```python
from build123d import *

# Parameters (mm, degrees)
BOSS_EXTRUDE1_DEPTH = 14
SKETCH3_W           = 2.1
SKETCH3_H           = 12.5


with BuildPart() as part:
    # Sketch1 → Boss-Extrude1 (new body)
    with BuildSketch(Plane.XY):
        with BuildLine():
            Line((-12.5, 25), (-12.5, 0))
            ThreePointArc((-12.5, 0), (0, -12.5), (12.5, 0))
            Line((12.5, 0), (12.5, 25))
            ThreePointArc((12.5, 25), (0, 37.5), (-12.5, 25))
        make_face()
        with BuildLine():
            Line((2.5, 9.9), (2.5, 7.177046746))
            ThreePointArc((2.5, 7.177046746), (6.195159401, 4.402272141), (7.6, 0))
            ThreePointArc((7.6, 0), (-4.402272141, -6.195159401), (-2.5, 7.177046746))
            Line((-2.5, 7.177046746), (-2.5, 9.9))
            Line((-2.5, 9.9), (2.5, 9.9))
        make_face(mode=Mode.SUBTRACT)
    extrude(amount=BOSS_EXTRUDE1_DEPTH)

    # Sketch3 → M5 Tapped Hole1 (revolve, cut)
    with BuildSketch(Plane(origin=(0, 0, 7), x_dir=(0, 0, 1), z_dir=(1, 0, 0))):
        with Locations((1.05, 6.25)):
            Rectangle(SKETCH3_W, SKETCH3_H)
    revolve(axis=Axis((0, 6.35, 7), (0, -1, 0)), mode=Mode.SUBTRACT)


solid = part.part
```
Geometry: final body of the model. Coordinates: model frame, mm. A direction names the side the tool comes from. Round coordinates to 2 decimals unless told otherwise and drop trailing zeros. Order: outer loops, then holes, each group sorted by start corner. A loop starts at its lowest first (then second) coordinate and runs counter-clockwise, first axis right, second up. Notation, with made-up numbers: (-18.5, 39) -> (35.5, 39) arc R23 ccw to (35.5, 77) -> close; hole circle Ø1 at (-9.75, -15.5). An arc over 180 degrees is marked (long way). Use CSV: the item, a comma, the result in double quotes. Start each with the question number.
1) Section D-D (y = -8.5). Return the cut outline in (x, z).
2) Draft query along X for faces 4 (the face through (0, 13, 14)), 5 (the face through (12.5, 12, 7)), 6 (the face through (0.275, 37.497, 6.902)), 7 (the face through (-2.5, 9, 7)). Return one class per face: +X half, -X half, draft (parallel to the pull), parting line (faces both ways), or undercut.
3) First-contact query: pin 1 Ø6 at (x, z) = (-7.5, 6.5) entering from +Y. Flat tip, straight axial feed; report the tip coordinate or a pass-through.
4) Set-up query: faces 1 (the face through (-0.09, -9.94, 4.9)), 2 (the face through (-0.275, -12.497, 10.013)), 3 (the face through (0, 9.9, 7)). Return all of +Z, -Z, +X, -X, +Y, -Y with unobstructed straight access to the full face (end or side cutting, diameter ignored); none if empty.
5) Section B-B (z = 13.25). Return the cut outline in (x, y), and give its area (3 significant figures).
6) Material intervals for line 1 along X through (y, z) = (0, 10); line 2 along Z through (x, y) = (0, -10.3); line 3 along X through (y, z) = (9.5, 9.75), sorted ascending. Write a range as from..to.
7) Section A-A (x = 0). Return the cut outline in (y, z), and give its area (3 significant figures).
8) Section C-C (x = -4.25). Return the cut outline in (y, z).
Returned:
1,outline,"(-9.17, 0) -> (9.17, 0) -> (9.17, 14) -> (-9.17, 14) -> close; hole circle Ø4.2 at (0, 7)"
2,face 4,"draft"
2,face 5,"+X half"
2,face 6,"parting line"
2,face 7,"undercut"
3,pin 1,"stops at y = 36.66"
4,face 1,"-Y"
4,face 2,"+Z, -Z, -Y"
4,face 3,"+Z, -Z"
5,outline,"(-12.5, 0) arc R12.5 ccw to (12.5, 0) -> (12.5, 25) arc R12.5 ccw to (-12.5, 25) -> close; hole (-2.5, 7.18) arc R7.6 ccw (long way) to (2.5, 7.18) -> (2.5, 9.9) -> (-2.5, 9.9) -> close"
5,area,"922 mm²"
6,line 1,"x = -12.5..-7.6, 7.6..12.5"
6,line 2,"z = 0..4.9, 9.1..14"
6,line 3,"x = -12.5..-2.5, 2.5..12.5"
7,outline,"(-12.5, 0) -> (-7.6, 0) -> (-7.6, 4.9) -> (-12.5, 4.9) -> close; (-12.5, 9.1) -> (-7.6, 9.1) -> (-7.6, 14) -> (-12.5, 14) -> close; (9.9, 0) -> (37.5, 0) -> (37.5, 14) -> (9.9, 14) -> close"
7,area,"434 mm²"
8,outline,"(-11.76, 0) -> (-6.3, 0) -> (-6.3, 14) -> (-11.76, 14) -> close; (6.3, 0) -> (36.76, 0) -> (36.76, 14) -> (6.3, 14) -> close"
